Source: CAD feature listing. Evaluate the final solid. Frame: model axes, mm. Face numbers are marked on the shaded views. A direction names the side the tool comes from. Round coordinates to 2 decimals unless told otherwise and drop trailing zeros. Order: outer loops, then holes, each group sorted by start corner. A loop starts at its lowest first (then second) coordinate and runs counter-clockwise, first axis right, second up. Notation, with made-up numbers: M 54.5,28 L 61.5,28 A25 cw 61.5,66 Z; hole C 0.5,-34.5 d9. An arc over 180 degrees is marked long. Answer as CSV lines item,"result". Start each with the question number.
Item 1: First-contact query: P1, Ø9.5, axis at x = 0, z = -46, coming from the +Y side; P2, Ø8.5, axis at x = 0, z = 0, coming from the +Y side; P3, Ø1, axis at x = -13, y = 5.5, coming from the -Z side. Flat tips, straight axial feed; report the tip coordinate or a pass-through.
Item 2: Section query D-D on z = -46. Return the cut outline in (x, y), plus the area to 3 significant figures.
Item 3: Section query A-A on x = 0. Return the cut outline in (y, z), plus the area to 3 significant figures.
Item 4: Set-up query: the marked faces 4 and 5. Return all of +Z, -Z, +X, -X, +Y, -Y with unobstructed straight access to the full face (end or side cutting, diameter ignored); none if empty.
Item 5: Pull-direction query (X, two-part tool) for the marked faces 1, 2 and 3; classes: +X half, -X half, draft (parallel to the pull), parting line (faces both ways), or undercut.
Item 6: Section query B-B on z = 0. Return the cut outline in (x, y).
Item 7: Section query C-C on y = 2. Return the cut outline in (x, z), plus the area to 3 significant figures.
Item 8: Line query: line 1 (X direction, y = 2.5, z = 0); line 2 (Z direction, x = 3, y = 8.75); line 3 (X direction, y = 8.6, z = -46). Output: solid intervals per line, ascending. Write a range as [from, to].
from build123d import *

# Parameters (mm, degrees)
SKETCH_1_W          = 60
SKETCH_1_H          = 120
EXTRUDE_1_DEPTH     = 10
SKETCH_2_R          = 8
CUT_EXTRUDE_1_DEPTH = 2
CHAMFER_1_SIZE      = 20
CUT_EXTRUDE_2_REACH = 69.823
SKETCH_3_R          = 5.25


with BuildPart() as part:
    # 草图1 → 凸台-拉伸1 (new body)
    with BuildSketch(Plane(origin=(0, 0, 0), x_dir=(1, 0, 0), z_dir=(0, 1, 0))):
        Rectangle(SKETCH_1_W, SKETCH_1_H)
    extrude(amount=EXTRUDE_1_DEPTH)

    # 草图2 → 切除-拉伸1 (cut)
    with BuildSketch(Plane(origin=(0, 10, 0), x_dir=(1, 0, 0), z_dir=(0, 1, 0))):
        with Locations(Location((0, 46, 0), (0, 0, 270))):
            Circle(SKETCH_2_R)
        with Locations(Location((0, -46, 0), (0, 0, 270))):
            Circle(SKETCH_2_R)
    extrude(amount=-CUT_EXTRUDE_1_DEPTH, mode=Mode.SUBTRACT)

    # 倒角1
    chamfer_1_edges = [part.edges().sort_by_distance(p)[0] for p in [
        (30, 5, 60),
        (-30, 5, 60),
        (-30, 5, -60),
        (30, 5, -60),
    ]]
    chamfer(chamfer_1_edges, length=CHAMFER_1_SIZE)

    # 草图3 → 切除-拉伸2 (cut, up to next)
    with BuildSketch(Plane(origin=(0, 10, 0), x_dir=(1, 0, 0), z_dir=(0, 1, 0)), mode=Mode.PRIVATE) as cut_extrude_2_sk1:
        with Locations(Location((0, 0, 0), (0, 0, 270))):
            Circle(SKETCH_3_R)
    cut_extrude_2_tool1 = extrude(cut_extrude_2_sk1.sketch, amount=-CUT_EXTRUDE_2_REACH, mode=Mode.PRIVATE) & part.part
    add(cut_extrude_2_tool1.solids().sort_by_distance((0, 10, 0))[0], mode=Mode.SUBTRACT)


solid = part.part
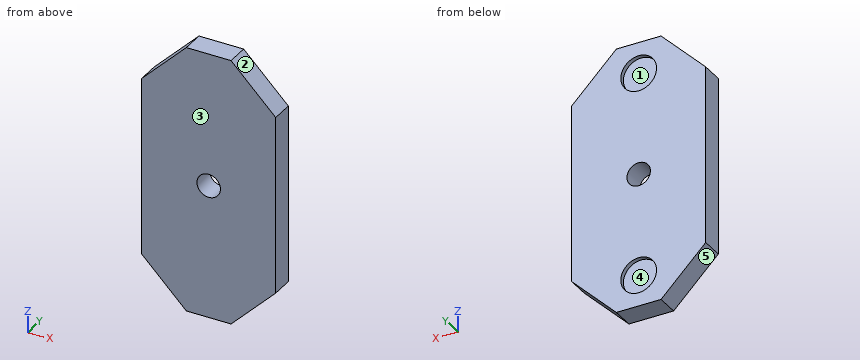
Results:
1,P1,"y = 8"
1,P2,"through"
1,P3,"z = -57.5"
2,outline,"M -24,0 L 24,0 L 24,10 L 8,10 L 8,8 L -8,8 L -8,10 L -24,10 Z"
2,area,"448 mm^2"
3,outline,"M 0,-60 L 10,-60 L 10,-54 L 8,-54 L 8,-38 L 10,-38 L 10,-5.25 L 0,-5.25 Z; M 0,5.25 L 10,5.25 L 10,38 L 8,38 L 8,54 L 10,54 L 10,60 L 0,60 Z"
3,area,"1,030 mm^2"
4,face 4,"+Y"
4,face 5,"-Z, -X, +Y, -Y"
5,face 1,"undercut"
5,face 2,"+X half"
5,face 3,"draft"
6,outline,"M -30,0 L -5.25,0 L -5.25,10 L -30,10 Z; M 5.25,0 L 30,0 L 30,10 L 5.25,10 Z"
7,outline,"M -30,-40 L -10,-60 L 10,-60 L 30,-40 L 30,40 L 10,60 L -10,60 L -30,40 Z; hole C 0,0 d10.5"
7,area,"6,310 mm^2"
8,line 1,"[-30, -5.25], [5.25, 30]"
8,line 2,"[-60, -53.42], [-38.58, -4.31], [4.31, 38.58], [53.42, 60]"
8,line 3,"[-24, -8], [8, 24]"
